Design review of the part built by this model. Coordinates are the model's own, in mm. Face numbers are marked on the shaded views. A direction names the side the tool comes from. Coordinates: 2 decimals unless noted, no trailing zeros. Loops run counter-clockwise (first coordinate to the right, second up) from the corner with the lowest first, then second, coordinate; pieces in that order, holes last. Notation, with made-up numbers: (35.25, 38) -> (45.25, 38) arc R28 cw to (45.25, 61) -> close; hole circle Ø7 at (59, -38). An arc over 180 degrees is marked (long way). Answer in a Markdown table with one row per item.
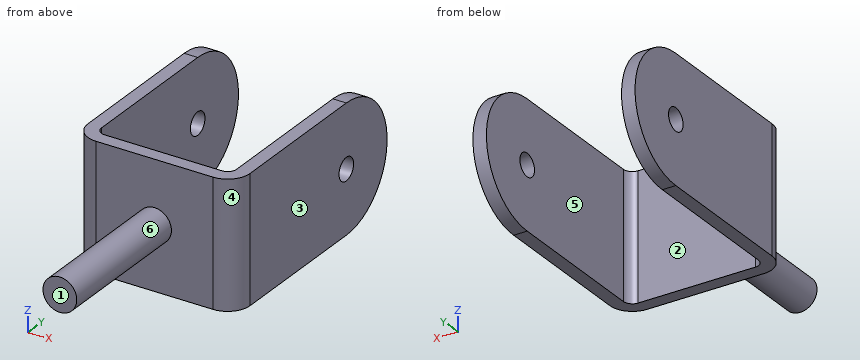
```python
from build123d import *

# Parameters (mm, degrees)
U_CHANNEL_BODY_DEPTH     = 140
STEM_SKETCH_75_R         = 37.5
STEM_75_DEPTH            = 325
UPRIGHT_TOP_ROUNDS_R50_R = 50
CHANNEL_FILLETS_R20_R    = 20
SIDE_BOSS_SKETCH_R       = 140
SIDE_BOSS_DEPTH          = 30
PIN_HOLE_SKETCH_R        = 25
PIN_HOLES_DEPTH          = 648.765389628


with BuildPart() as part:
    # U-Channel Profile Sketch → U-Channel Body (new, symmetric)
    with BuildSketch(Plane.XY):
        Polygon((-180, 380), (-180, 0), (180, 0), (180, 380), (150, 380), (150, 30), (-150, 30), (-150, 380), align=None)
    extrude(amount=U_CHANNEL_BODY_DEPTH, both=True)

    # Stem Sketch Ø75 → Stem Ø75 (add)
    with BuildSketch(Plane.XZ):
        Circle(STEM_SKETCH_75_R)
    extrude(amount=STEM_75_DEPTH)

    # Upright Top Rounds R50
    upright_top_rounds_r50_edges = [part.edges().sort_by_distance(p)[0] for p in [
        (180, 0, 0),
        (-180, 0, 0),
    ]]
    fillet(upright_top_rounds_r50_edges, radius=UPRIGHT_TOP_ROUNDS_R50_R)

    # Channel Fillets R20
    channel_fillets_r20_edges = [part.edges().sort_by_distance(p)[0] for p in [
        (-150, 30, 0),
        (150, 30, 0),
    ]]
    fillet(channel_fillets_r20_edges, radius=CHANNEL_FILLETS_R20_R)

    # Side Boss Sketch → Side Boss (add)
    with BuildSketch(Plane(origin=(180, 0, 0), x_dir=(0, 0, -1), z_dir=(1, 0, 0))):
        with Locations((0, 380)):
            Circle(SIDE_BOSS_SKETCH_R)
    side_boss = extrude(amount=-SIDE_BOSS_DEPTH)

    # Side Boss Mirror: Side Boss across plane
    add(side_boss.mirror(Plane(origin=(0, 0, 0), x_dir=(0, 0, 1), z_dir=(1, 0, 0))))

    # Pin Hole Sketch → Pin Holes (cut, through all)
    with BuildSketch(Plane.ZY.offset(180)):
        with Locations(Location((0, 380, 0), (0, 0, 270))):
            Circle(PIN_HOLE_SKETCH_R)
    extrude(amount=-PIN_HOLES_DEPTH, mode=Mode.SUBTRACT)


solid = part.part
```
(1) Take a section at B-B on y = 94. Give the boundary of the cut face in (x, z), and give its area (3 significant figures).
Evaluation:
| item | result |
|---|---|
| outline | (-180, -140) -> (-150, -140) -> (-150, 140) -> (-180, 140) -> close; (150, -140) -> (180, -140) -> (180, 140) -> (150, 140) -> close |
| area | 16,800 mm² |
(2) Take a section at C-C on x = 22.5. Give the boundary of the cut face in (y, z), and give its area (3 significant figures).
Evaluation:
| item | result |
|---|---|
| outline | (-325, -30) -> (0, -30) -> (0, -140) -> (30, -140) -> (30, 140) -> (0, 140) -> (0, 30) -> (-325, 30) -> close |
| area | 27,900 mm² |
(3) Take a section at D-D on z = 117. Give the boundary of the cut face in (x, y), and give its area (3 significant figures).
Evaluation:
| item | result |
|---|---|
| outline | (-180, 50) arc R50 ccw to (-130, 0) -> (130, 0) arc R50 ccw to (180, 50) -> (180, 456.88) -> (150, 456.88) -> (150, 50) arc R20 cw to (130, 30) -> (-130, 30) arc R20 cw to (-150, 50) -> (-150, 456.88) -> (-180, 456.88) -> close |
| area | 35,500 mm² |
(4) Take a section at A-A on z = 0. Give the boundary of the cut face in (x, y).
Evaluation:
| item | result |
|---|---|
| outline | (-180, 50) arc R50 ccw to (-130, 0) -> (-37.5, 0) -> (-37.5, -325) -> (37.5, -325) -> (37.5, 0) -> (130, 0) arc R50 ccw to (180, 50) -> (180, 355) -> (150, 355) -> (150, 50) arc R20 cw to (130, 30) -> (-130, 30) arc R20 cw to (-150, 50) -> (-150, 355) -> (-180, 355) -> close; (-180, 405) -> (-150, 405) -> (-150, 520) -> (-180, 520) -> close; (150, 405) -> (180, 405) -> (180, 520) -> (150, 520) -> close |
(5) For pin 1 (12 mm diameter, centred on y = -140, z = 14.5, fed in from +X); pin 2 (8 mm diameter, centred on y = -67, z = -34, fed in from +X); pin 3 (1 mm diameter, centred on x = -112.5, z = -92, fed in from +Y), all flat-tipped, find the tip position at first contact; note any pin that passes through.
Evaluation:
| item | result |
|---|---|
| pin 1 | stops at x = 36.52 |
| pin 2 | stops at x = 22.5 |
| pin 3 | stops at y = 30 |
(6) To check wall thickness, follow probe 1 along Z at (x, y) = (-166, 380); probe 2 along X at (y, z) = (236, 16); probe 3 along Y at (x, z) = (-72.5, -59.5). State the ranges of each line that lie inside material, in increasing order.
Evaluation:
| item | result |
|---|---|
| probe 1 | z = -140 to -25, 25 to 140 |
| probe 2 | x = -180 to -150, 150 to 180 |
| probe 3 | y = 0 to 30 |
(7) Draft analysis for pull direction X (two halves, no side actions). For the marked faces 1, 2 and 3, state which applies: pulls with the +X half, pulls with the -X half, needs draft (parallel to the pull), parting line crosses it, or undercut.
Evaluation:
| item | result |
|---|---|
| face 1 | needs draft |
| face 2 | undercut |
| face 3 | pulls with the +X half |
(8) Tool access review of the marked faces 4, 5 and 6: name each direction out of +Z, -Z, +X, -X, +Y, -Y from which nothing blocks a thin tool from reaching the whole face with its end or side.
Evaluation:
| item | result |
|---|---|
| face 4 | +Z, -Z, +X, -Y |
| face 5 | +Z, -Z, +Y |
| face 6 | -Y |
